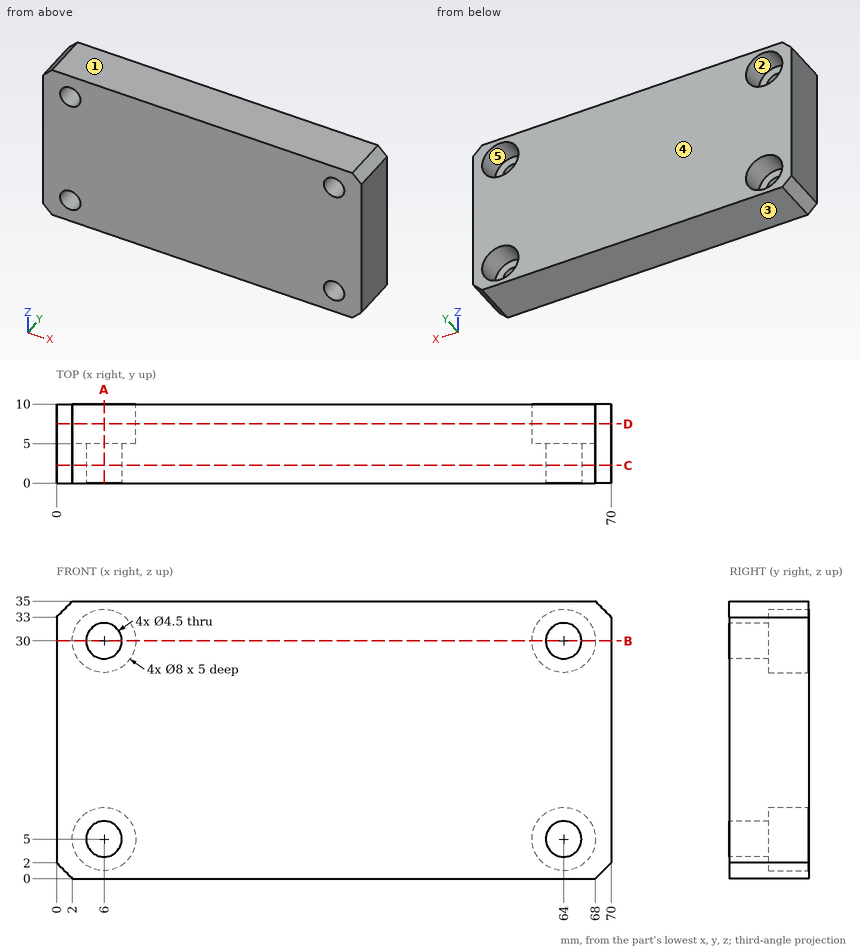
Source: three-view drawing plus pictorial views. Frame: mm from the lowest corner of the part. A direction names the side the tool comes from. Round coordinates to 2 decimals unless told otherwise and drop trailing zeros. Write each loop counter-clockwise with the first axis right and the second up, starting at its lowest first coordinate (ties: lowest second). Pieces come first, ordered by that corner, then holes. Notation, with made-up numbers: M 9.25,13.25 L 24.25,13.25 A19 ccw 24.25,27.25 Z; hole C 24,-34 d8. An arc over 180 degrees is marked long. Write item = value, one per line.
Item 1: Access query for the marked faces 1 and 2. Directions: +Z, -Z, +X, -X, +Y, -Y. A direction counts if a zero-diameter tool reaches every point of the face in a straight line with its end or side. Return the directions, or none.
Findings:
face_1 = +Z, +X, -X, +Y, -Y
face_2 = +Y
Item 2: Section query C-C on y = 2.25. Return loops of the section in (x, z).
Findings:
outline = M 0,2 L 2,0 L 68,0 L 70,2 L 70,33 L 68,35 L 2,35 L 0,33 Z; hole C 6,5 d4.5; hole C 6,30 d4.5; hole C 64,5 d4.5; hole C 64,30 d4.5
Item 3: Material intervals for line 1 along Z through (x, y) = (64, 6.7); line 2 along X through (y, z) = (8.7, 30); line 3 along Z through (x, y) = (6, 3.85), sorted ascending. Write a range as [from, to].
Findings:
line_1 = [0, 1], [9, 26], [34, 35]
line_2 = [0, 2], [10, 60], [68, 70]
line_3 = [0, 2.75], [7.25, 27.75], [32.25, 35]
Item 4: Pin query (flat end, axial travel): P1, Ø4, axis at x = 7, z = 5.5, coming from the +Y side; P2, Ø3.5, axis at x = 6, z = 5, coming from the -Y side. Return the tip coordinate at first contact, or that it passes through.
Findings:
P1 = 5
P2 = through
Item 5: Section query A-A on x = 6. Return loops of the section in (y, z).
Findings:
outline = M 0,0 L 10,0 L 10,1 L 5,1 L 5,2.75 L 0,2.75 Z; M 0,7.25 L 5,7.25 L 5,9 L 10,9 L 10,26 L 5,26 L 5,27.75 L 0,27.75 Z; M 0,32.25 L 5,32.25 L 5,34 L 10,34 L 10,35 L 0,35 Z
Item 6: Section query B-B on z = 30. Return loops of the section in (x, y).
Findings:
outline = M 0,0 L 3.75,0 L 3.75,5 L 2,5 L 2,10 L 0,10 Z; M 8.25,0 L 61.75,0 L 61.75,5 L 60,5 L 60,10 L 10,10 L 10,5 L 8.25,5 Z; M 66.25,0 L 70,0 L 70,10 L 68,10 L 68,5 L 66.25,5 Z
Item 7: Pull-direction query (Z, two-part tool) for the marked faces 3, 4 and 5; classes: pulls with the +Z half, pulls with the -Z half, needs draft (parallel to the pull), parting line crosses it, or undercut.
Findings:
face_3 = pulls with the -Z half
face_4 = needs draft
face_5 = undercut
Item 8: Section query D-D on y = 7.5. Return loops of the section in (x, z).
Findings:
outline = M 0,2 L 2,0 L 68,0 L 70,2 L 70,33 L 68,35 L 2,35 L 0,33 Z; hole C 6,5 d8; hole C 6,30 d8; hole C 64,5 d8; hole C 64,30 d8
